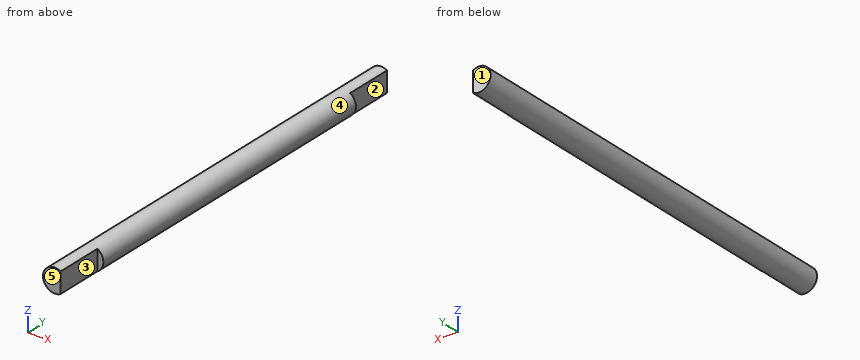
```python
from build123d import *

# Parameters (mm, degrees)
SKETCH_1_R          = 15
EXTRUDE_1_DEPTH     = 531
CUT_EXTRUDE_START   = -60
CUT_EXTRUDE_1_DEPTH = 60


with BuildPart() as part:
    # 草图1 → 凸台-拉伸1 (new body)
    with BuildSketch(Plane(origin=(0, 0, 0), x_dir=(1, 0, 0), z_dir=(0, 1, 0))):
        with Locations(Location((0, 0, 0), (0, 0, 270))):
            Circle(SKETCH_1_R)
    extrude(amount=EXTRUDE_1_DEPTH)

    # 草图2 → 切除-拉伸1 (cut)
    with BuildSketch(Plane(origin=(0, 531, 0), x_dir=(1, 0, 0), z_dir=(0, 1, 0)).offset(CUT_EXTRUDE_START)):
        with BuildLine():
            Line((7.5, 12.990381057), (7.5, -12.990381057))
            ThreePointArc((7.5, -12.990381057), (15, 0), (7.5, 12.990381057))
        make_face()
    cut_extrude_1 = extrude(amount=CUT_EXTRUDE_1_DEPTH, mode=Mode.SUBTRACT)

    # 镜向1: 切除-拉伸1 across plane
    add(cut_extrude_1.mirror(Plane.ZX.offset(265.5)), mode=Mode.SUBTRACT)


solid = part.part
```
Could you check a few things on this model? Use its own coordinates, in mm. Face numbers are marked on the shaded views. A direction names the side the tool comes from. Give positions to 0.01 mm unless a question says otherwise; leave off trailing zeros. Order: outer loops, then holes, each group sorted by start corner. A loop starts at its lowest first (then second) coordinate and runs counter-clockwise, first axis right, second up.
Q1. For the marked faces 1 and 2, which set-ups out of +Z, -Z, +X, -X, +Y, -Y let a thin tool reach every point of the face, with its end or its side?
Q2. Suppose I cut it at B-B, the plane y = 276. Write out the boundary of the cut face in (x, z).
Q3. If I drill on line 1 along Y through (x, z) = (9, -7.75); line 2 along X through (y, z) = (164, -7.5); line 3 along Z through (x, y) = (-1, 479), over which ranges is the centre line in solid material (lowest first)?
Q4. Suppose I cut it at A-A, the plane z = 0. Write out the boundary of the cut face in (x, y).
Q5. Suppose I cut it at C-C, the plane x = -8.5. Write out the boundary of the cut face in (y, z).
Q6. I'm going to push flat-ended pins straight in: P1, Ø1.5, axis at x = 10, y = 98, coming from the -Z side; P2, Ø8, axis at y = 506.5, z = 0.5, coming from the +X side; P3, Ø1.5, axis at x = 7, y = 152, coming from the -Z side. Where does each tip first touch, or does it pass through?
Q7. We'd pull the mould along X, two halves only. Please class the marked faces 3, 4 and 5: +X half, -X half, draft (parallel to the pull), parting line (faces both ways), or undercut.
Solution:
1. face 1: +Z, -Z, +X, -X, +Y
1. face 2: +Z, -Z, +X, +Y
2. outline: circle Ø30 at (0, 0)
3. line 1: y = 60 to 471
3. line 2: x = -12.99 to 12.99
3. line 3: z = -14.97 to 14.97
4. outline: (-15, 0) - (7.5, 0) - (7.5, 60) - (15, 60) - (15, 471) - (7.5, 471) - (7.5, 531) - (-15, 531) - close
5. outline: (0, -12.36) - (531, -12.36) - (531, 12.36) - (0, 12.36) - close
6. P1: stops at z = -11.81
6. P2: stops at x = 7.5
6. P3: stops at z = -13.64
7. face 3: +X half
7. face 4: parting line
7. face 5: draft
